CAD build for the part. Positions are in the model's coordinates, mm. A direction names the side the tool comes from. Round coordinates to 2 decimals unless told otherwise and drop trailing zeros. Write each loop counter-clockwise with the first axis right and the second up, starting at its lowest first coordinate (ties: lowest second). Pieces come first, ordered by that corner, then holes. Notation, with made-up numbers: (1, 69.5) -> (22, 69.5) arc R12 cw to (22, 84.5) -> close; hole circle Ø8 at (57.25, 29.5). An arc over 180 degrees is marked (long way). Answer in a Markdown table with one row per item. Add a question column.
```python
from build123d import *

# Parameters (mm, degrees)
SKETCH_1_W             = 51
SKETCH_1_H             = 73
EXTRUDE_1_DEPTH        = 26
FILLET_1_R             = 5
SKETCH_2_W             = 5
SKETCH_2_H             = 5
CUT_EXTRUDE_1_DEPTH    = 30
HOLE_WIZARD_M3_1_D     = 2.5
HOLE_WIZARD_M3_1_DEPTH = 7.5
HOLE_WIZARD_M3_1_TIP   = 0.751075774


with BuildPart() as part:
    # 草图1 → 凸台-拉伸1 (new body)
    with BuildSketch(Plane(origin=(0, 0, 0), x_dir=(1, 0, 0), z_dir=(0, 1, 0))):
        Rectangle(SKETCH_1_W, SKETCH_1_H)
    extrude(amount=EXTRUDE_1_DEPTH)

    # 圆角1
    fillet_1_edges = [part.edges().sort_by_distance(p)[0] for p in [
        (25.5, 13, 36.5),
        (-25.5, 13, 36.5),
        (-25.5, 13, -36.5),
        (25.5, 13, -36.5),
    ]]
    fillet(fillet_1_edges, radius=FILLET_1_R)

    # 草图2 → 切除-拉伸1 (cut)
    with BuildSketch(Plane.XZ):
        with Locations((23, -34)):
            Rectangle(SKETCH_2_W, SKETCH_2_H)
        with Locations((-23, -34)):
            Rectangle(SKETCH_2_W, SKETCH_2_H)
    extrude(amount=-CUT_EXTRUDE_1_DEPTH, mode=Mode.SUBTRACT)

    # M3 螺纹孔1
    with Locations(Plane(origin=(0, 0, 0), x_dir=(-1, 0, 0), z_dir=(0, -1, 0))):
        with Locations((14.8, -8.3), (-16.2, -8.3), (14.8, 21.7), (-16.2, 21.7)):
            Hole(HOLE_WIZARD_M3_1_D / 2, depth=HOLE_WIZARD_M3_1_DEPTH)
            with Locations((0, 0, -(HOLE_WIZARD_M3_1_DEPTH + HOLE_WIZARD_M3_1_TIP / 2))):  # 118° drill point
                Cone(0, HOLE_WIZARD_M3_1_D / 2, HOLE_WIZARD_M3_1_TIP, mode=Mode.SUBTRACT)


solid = part.part
```
Item 1: Drill centre lines: probe 1 along Z at (x, y) = (-14.8, 3.5); probe 2 along X at (y, z) = (2.5, 8.3); probe 3 along X at (y, z) = (19.5, 33). Where is each one in solid material? Low to high.
Item 2: Saw through at A-A on y = 6. Give the cut face in (x, z), then the cut area to 3 significant figures.
Item 3: Tool access for faces 4 (the flat face through (0, 0, -1)), 5 (the cylindrical face through (-14.128, 3.802, -22.754)), 6 (the flat face through (-23, 13, -31.5)), 7 (the flat face through (23, 13, -31.5)): list every direction of +Z, -Z, +X, -X, +Y, -Y with a clear straight run to the whole face (end or side of a thin tool).
Item 4: Two-plate mould, pull along Z, no slides. Class faces 1 (the cylindrical face through (17.355, 3.802, 8.779)), 2 (the cylindrical face through (24, 13.18, 35.07)), 3 (the flat face through (25.5, 13, 0)): +Z half, -Z half, draft (parallel to the pull), parting line (faces both ways), or undercut.
Item 5: Pin check, flat tips, straight feed: pin 1 (1.5 mm diameter, centred on x = -24, y = 13, fed in from -Z); pin 2 (2 mm diameter, centred on x = 16.2, z = -21.7, fed in from -Y); pin 3 (1.5 mm diameter, centred on y = 16.5, z = -35, fed in from -X). Stop position of each tip, or through.
Item 6: Saw through at C-C on x = 21.5. Give the cut face in (y, z).
Item 7: Saw through at B-B on y = 16. Give the cut face in (x, z).
Recorded:
| question | item | result |
|---|---|---|
| 1 | probe 1 | -36.5 to -22.95, -20.45 to 7.05, 9.55 to 36.5 |
| 1 | probe 2 | -25.5 to -16.05, -13.55 to 14.95, 17.45 to 25.5 |
| 1 | probe 3 | -25.27 to 25.27 |
| 2 | outline | (-25.5, -31.5) -> (-20.5, -31.5) -> (-20.5, -36.5) -> (20.5, -36.5) -> (20.5, -31.5) -> (25.5, -31.5) -> (25.5, 31.5) arc R5 ccw to (20.5, 36.5) -> (-20.5, 36.5) arc R5 ccw to (-25.5, 31.5) -> close; hole circle Ø2.5 at (-14.8, -21.7); hole circle Ø2.5 at (-14.8, 8.3); hole circle Ø2.5 at (16.2, -21.7); hole circle Ø2.5 at (16.2, 8.3) |
| 2 | area | 3,640 mm2 |
| 3 | face 4 | +Z, -Z, +X, -X, -Y |
| 3 | face 5 | -Y |
| 3 | face 6 | -Z, -X, +Y, -Y |
| 3 | face 7 | -Z, +X, +Y, -Y |
| 4 | face 1 | undercut |
| 4 | face 2 | +Z half |
| 4 | face 3 | draft |
| 5 | pin 1 | z = -31.5 |
| 5 | pin 2 | y = 7.65 |
| 5 | pin 3 | x = -20.5 |
| 6 | outline | (0, -31.5) -> (26, -31.5) -> (26, 36.4) -> (0, 36.4) -> close |
| 7 | outline | (-25.5, -31.5) -> (-20.5, -31.5) -> (-20.5, -36.5) -> (20.5, -36.5) -> (20.5, -31.5) -> (25.5, -31.5) -> (25.5, 31.5) arc R5 ccw to (20.5, 36.5) -> (-20.5, 36.5) arc R5 ccw to (-25.5, 31.5) -> close |
